The listing builds one solid part. Answer for the finished solid, in the listing's coordinates (mm). A direction names the side the tool comes from. Round coordinates to 2 decimals unless told otherwise and drop trailing zeros. One line per question, with ' | ' between items.
from build123d import *

# Parameters (mm, degrees)
SKETCH_1_W                = 665
SKETCH_1_H                = 20
EXTRUDE_1_DEPTH           = 15
HOLE_WIZARD_1_D           = 6.6
HOLE_WIZARD_1_CBORE_D     = 11
HOLE_WIZARD_1_CBORE_DEPTH = 6.8


with BuildPart() as part:
    # 草图1 → 凸台-拉伸1 (new body)
    with BuildSketch(Plane.XY):
        Rectangle(SKETCH_1_W, SKETCH_1_H)
    extrude(amount=EXTRUDE_1_DEPTH)

    # 打孔尺寸(%根据)内六角圆柱头螺钉的类型1 (through all)
    with Locations(Plane.XY.offset(15)):
        with Locations((102.5, 0), (-307.5, 0), (307.5, 0), (-102.5, 0)):
            CounterBoreHole(HOLE_WIZARD_1_D / 2, HOLE_WIZARD_1_CBORE_D / 2, HOLE_WIZARD_1_CBORE_DEPTH)


solid = part.part
Q1. A cutting plane is placed at A-A on y = 0. Give the number of separate pieces and of enclosed holes in the cut face, plus the area to 3 significant figures.
Numbers:
separate pieces: 5 | enclosed holes: 0 | area: 9,460 mm^2
Q2. Given pin 1 Ø12 at (x, y) = (310, 1.5) entering from +Z; pin 2 Ø5.5 at (x, y) = (103.5, 0) entering from +Z, each flat-ended and moving along its own axis, determine where each tip first touches the part or whether it passes through.
Numbers:
pin 1: z = 15 | pin 2: z = 8.2
Q3. For a pull along X with two mould halves and no side action, classify faces 1 (the face through (332.5, 0, 7)), 2 (the face through (-5, -10, 7)), 3 (the face through (97, 0, 12)) as pulls with the +X half, pulls with the -X half, needs draft (parallel to the pull), parting line crosses it, or undercut.
Numbers:
face 1: pulls with the +X half | face 2: needs draft | face 3: undercut
Q4. For faces 4 (the face through (-5, 0, 0)), 5 (the face through (-99, 0, 8.2)), determine the directions among +Z, -Z, +X, -X, +Y, -Y from which every point of the face is accessible in a straight line to the end or side of a thin tool.
Numbers:
face 4: -Z, +X, -X, +Y, -Y | face 5: +Z
Q5. Find the intervals of material crossed by line 1 (Y direction, x = -307.5, z = 13); line 2 (Y direction, x = -307.5, z = 1.5), in increasing order. Write a range as from..to.
Numbers:
line 1: -10..-5.5, 5.5..10 | line 2: -10..-3.3, 3.3..10
